For this review, take the finished solid that the model builds, in its own axes (mm). A direction names the side the tool comes from. Give positions to 0.01 mm unless a question says otherwise; leave off trailing zeros. Order: outer loops, then holes, each group sorted by start corner. A loop starts at its lowest first (then second) coordinate and runs counter-clockwise, first axis right, second up. Notation, with made-up numbers: (89.5, 0.5) - (97.5, 0.5) arc R24 ccw to (97.5, 30.5) - close; hole circle Ø4 at (17.25, 22.5). An arc over 180 degrees is marked (long way). Use a Markdown table: item, result. Add a question column.
1) We need section C-C on x = -14. Write out the cut boundary in (y, z).
2) We need section A-A on y = -1. Write out the cut boundary in (x, z).
3) Wall thickness on L1, parallel to Y at x = 27.5, z = -1.6; L2, parallel to X at y = 1.5, z = -3.5; L3, parallel to Y at x = -27, z = -3.5: over which ranges is each line inside the solid? List them lowest first.
4) Mouldability with a two-part tool opening along X and no side actions: class faces 4 (the face through (-9.666, -33.278, 0.07)), 5 (the face through (-40, 0, 0)), 6 (the face through (8, 1, 5)) as released by +X, released by -X, zero draft, split by the parting line, or undercut.
5) Clearance check with a flat-ended pin moving along its axis: P1, Ø5, axis at x = 28.5, y = 25.5, coming from the -Z side. State where the tip first meets the part, or that it passes through.
6) We need section D-D on y = -32. Write out the cut boundary in (x, z).
7) Machinability: for faces 1 (the face through (25, -27, 0.7)), 2 (the face through (-1, 37.5, 0)), 3 (the face through (-17, 25, 0)), which of the approach directions +Z, -Z, +X, -X, +Y, -Y give a long, thin tool a straight path to every point of the face, cutting with its end or side? Answer none if there is none.
8) We need section B-B on z = 2. Write out the cut boundary in (x, y).
```python
from build123d import *

# Parameters (mm, degrees)
SKETCH_1_W                   = 80
SKETCH_1_H                   = 75
EXTRUDE_1_DEPTH              = 5
CHAMFER_1_SIZE               = 2
HOLE_WIZARD_M5_1_D           = 5.5
HOLE_WIZARD_M5_1_CBORE_D     = 10
HOLE_WIZARD_M5_1_CBORE_DEPTH = 5.7
HOLE_WIZARD_M5_1_2_D         = 4.2
HOLE_WIZARD_M5_1_2_DEPTH     = 12.4
HOLE_WIZARD_M5_1_2_TIP       = 1.2618073
CUT_EXTRUDE_1_DEPTH          = 56.733742024


with BuildPart() as part:
    # 草图1 → 凸台-拉伸1 (new, symmetric)
    with BuildSketch(Plane.XY):
        Rectangle(SKETCH_1_W, SKETCH_1_H)
    extrude(amount=EXTRUDE_1_DEPTH, both=True)

    # 倒角1
    chamfer_1_edges = [part.edges().sort_by_distance(p)[0] for p in [
        (40, -37.5, 0),
        (-40, -37.5, 0),
        (-40, 37.5, 0),
        (40, 37.5, 0),
    ]]
    chamfer(chamfer_1_edges, length=CHAMFER_1_SIZE)

    # Hole Wizard M5 _1 (through all)
    with Locations(Plane(origin=(0, 0, -5), x_dir=(-1, 0, 0), z_dir=(0, 0, -1))):
        with Locations((-27.5, 25), (-27.5, -25)):
            CounterBoreHole(HOLE_WIZARD_M5_1_D / 2, HOLE_WIZARD_M5_1_CBORE_D / 2, HOLE_WIZARD_M5_1_CBORE_DEPTH)

    # Hole Wizard M5 _1 2
    with Locations(Plane(origin=(0, 0, -5), x_dir=(-1, 0, 0), z_dir=(0, 0, -1))):
        with Locations((7.999483419, 32), (25.999483419, 32), (7.999483419, -32), (25.999483419, -32)):
            Hole(HOLE_WIZARD_M5_1_2_D / 2, depth=HOLE_WIZARD_M5_1_2_DEPTH)
            with Locations((0, 0, -(HOLE_WIZARD_M5_1_2_DEPTH + HOLE_WIZARD_M5_1_2_TIP / 2))):  # 118° drill point
                Cone(0, HOLE_WIZARD_M5_1_2_D / 2, HOLE_WIZARD_M5_1_2_TIP, mode=Mode.SUBTRACT)

    # 草图8 → 切除-拉伸1 (cut, through all)
    with BuildSketch(Plane(origin=(0, 0, -5), x_dir=(-1, 0, 0), z_dir=(0, 0, -1))):
        with BuildLine():
            Line((9.499483419, -25), (24.499483419, -25))
            ThreePointArc((24.499483419, -25), (28.035017325, -23.535533906), (29.499483419, -20))
            Line((29.499483419, -20), (29.499483419, 20))
            ThreePointArc((29.499483419, 20), (28.035017325, 23.535533906), (24.499483419, 25))
            Line((24.499483419, 25), (9.499483419, 25))
            ThreePointArc((9.499483419, 25), (5.963949513, 23.535533906), (4.499483419, 20))
            Line((4.499483419, 20), (4.499483419, -20))
            ThreePointArc((4.499483419, -20), (5.963949513, -23.535533906), (9.499483419, -25))
        make_face()
    extrude(amount=-CUT_EXTRUDE_1_DEPTH, mode=Mode.SUBTRACT)


solid = part.part
```
Checked values:
| question | item | result |
|---|---|---|
| 1 | outline | (-37.5, -5) - (-25, -5) - (-25, 5) - (-37.5, 5) - close; (25, -5) - (37.5, -5) - (37.5, 5) - (25, 5) - close |
| 2 | outline | (-40, -5) - (-29.5, -5) - (-29.5, 5) - (-40, 5) - close; (-4.5, -5) - (40, -5) - (40, 5) - (-4.5, 5) - close |
| 3 | L1 | -37.5 to -30, -20 to 20, 30 to 37.5 |
| 3 | L2 | -40 to -29.5, -4.5 to 40 |
| 3 | L3 | -37.5 to -33.85, -30.15 to -24.33, 24.33 to 30.15, 33.85 to 37.5 |
| 4 | face 4 | undercut |
| 4 | face 5 | released by -X |
| 4 | face 6 | zero draft |
| 5 | P1 | z = 0.7 |
| 6 | outline | (-40, -5) - (-28.1, -5) - (-28.1, 5) - (-40, 5) - close; (-23.9, -5) - (-10.1, -5) - (-10.1, 5) - (-23.9, 5) - close; (-5.9, -5) - (40, -5) - (40, 5) - (-5.9, 5) - close |
| 7 | face 1 | -Z |
| 7 | face 2 | +Z, -Z, +X, -X, +Y |
| 7 | face 3 | +Z, -Z |
| 8 | outline | (-40, -35.5) - (-38, -37.5) - (38, -37.5) - (40, -35.5) - (40, 35.5) - (38, 37.5) - (-38, 37.5) - (-40, 35.5) - close; hole (-29.5, -20) arc R5 ccw to (-24.5, -25) - (-9.5, -25) arc R5 ccw to (-4.5, -20) - (-4.5, 20) arc R5 ccw to (-9.5, 25) - (-24.5, 25) arc R5 ccw to (-29.5, 20) - close; hole circle Ø4.2 at (-26, -32); hole circle Ø4.2 at (-26, 32); hole circle Ø4.2 at (-8, -32); hole circle Ø4.2 at (-8, 32); hole circle Ø5.5 at (27.5, -25); hole circle Ø5.5 at (27.5, 25) |
